Build history of the part. All positions in model axes, mm. Face numbers are marked on the shaded views. A direction names the side the tool comes from. Give positions to 0.01 mm unless a question says otherwise; leave off trailing zeros. Loops run counter-clockwise (first coordinate to the right, second up) from the corner with the lowest first, then second, coordinate; pieces in that order, holes last. Notation, with made-up numbers: (85, 52) -> (141, 52) arc R29 ccw to (141, 81) -> close; hole circle Ø2 at (21, 65.5). An arc over 180 degrees is marked (long way). Answer as a JSON object with one key per item and string values. Group by question number.
Q1. Wall check: probe 1 along X at (y, z) = (-6, 82.5); probe 2 along X at (y, z) = (-10, 86.5). Give the ranges that are in metal, low to high. Write a range as from..to.
Q2. Drop flat-ended pins along their axis: pin 1 (12 mm diameter, centred on y = -4, z = 67.5, fed in from -X); pin 2 (3 mm diameter, centred on y = 5.5, z = 223, fed in from +X); pin 3 (1.2 mm diameter, centred on x = 12, y = -0.5, fed in from +Z). Give the stop position or say it passes through.
Q3. Tool access for the marked faces 1, 2 and 3: list every direction of +Z, -Z, +X, -X, +Y, -Y with a clear straight run to the whole face (end or side of a thin tool).
Q4. Band-saw the part on A-A, the plane z = 61. Write the cut outline in (x, y), plus the area to 3 significant figures.
from build123d import *

# Parameters (mm, degrees)
SKETCH5_OUTSIDE_W  = 88.64
SKETCH5_OUTSIDE_H  = 88.64
CUT_EXTRUDE1_DEPTH = 18
SKETCH6_OUTSIDE_W  = 123.2
SKETCH6_OUTSIDE_H  = 119.18
SKETCH6_OUTSIDE_R  = 12.990381057
CUT_EXTRUDE2_DEPTH = 10
CUT_EXTRUDE2_DRAFT = -60
SKETCH7_OUTSIDE_W  = 123.2
SKETCH7_OUTSIDE_H  = 119.18
SKETCH7_OUTSIDE_R  = 12.990381057
CUT_EXTRUDE3_DEPTH = 10
CUT_EXTRUDE3_DRAFT = -60
SKETCH9_W          = 22
SKETCH9_H          = 25.980762114
CUT_EXTRUDE4_DEPTH = 7
CHAMFER1_SIZE      = 1


with BuildPart() as part:
    # Sketch3 → Revolve1 (revolve)
    with BuildSketch(Plane(origin=(0, 0, 0), x_dir=(0, 0, -1), z_dir=(1, 0, 0)), mode=Mode.PRIVATE) as revolve1_sk:
        Polygon((-38, 12.5), (-38, 0), (-318, 0), (-318, 10), (-299, 10), (-299, 15), (-281, 15), (-281, 10), (-278, 10), (-278, 12.5), align=None)
    revolve(revolve1_sk.sketch.rotate(Axis((0, 0, 318), (0, 0, -1)), 180), axis=Axis((0, 0, 318), (0, 0, -1)))

    # Sketch5 outside → Cut-Extrude1 (cut)
    with BuildSketch(Plane.XY.offset(299)):
        Rectangle(SKETCH5_OUTSIDE_W, SKETCH5_OUTSIDE_H)
        Polygon((7.5, 12.990381057), (-7.5, 12.990381057), (-15, 0), (-7.5, -12.990381057), (7.5, -12.990381057), (15, 0), align=None, mode=Mode.SUBTRACT)
    extrude(amount=-CUT_EXTRUDE1_DEPTH, mode=Mode.SUBTRACT)


with BuildPart() as cut_extrude2_tool:
    # Sketch6 outside → Cut-Extrude2 (with draft: the straight prism first)
    with BuildSketch(Plane.XY.offset(299)):
        Rectangle(SKETCH6_OUTSIDE_W, SKETCH6_OUTSIDE_H)
        Circle(SKETCH6_OUTSIDE_R, mode=Mode.SUBTRACT)
    extrude(amount=-CUT_EXTRUDE2_DEPTH)
    # Cut-Extrude2: the draft: its side faces are tilted about the plane it starts from
    cut_extrude2_sides = [cut_extrude2_tool.faces().sort_by_distance(p)[0] for p in [
        (0, -59.59, 294),
        (61.6, 0, 294),
        (0, 59.59, 294),
        (-61.6, 0, 294),
        (-12.990381057, 0, 294),
    ]]
    draft(cut_extrude2_sides, Plane.XY.offset(299), CUT_EXTRUDE2_DRAFT)


with BuildPart() as part_1:
    add(part.part)

    # Cut-Extrude2: cut by cut_extrude2_tool
    add(cut_extrude2_tool.part, mode=Mode.SUBTRACT)


with BuildPart() as cut_extrude3_tool:
    # Sketch7 outside → Cut-Extrude3 (with draft: the straight prism first)
    with BuildSketch(Plane(origin=(0, 0, 281), x_dir=(-1, 0, 0), z_dir=(0, 0, -1))):
        Rectangle(SKETCH7_OUTSIDE_W, SKETCH7_OUTSIDE_H)
        Circle(SKETCH7_OUTSIDE_R, mode=Mode.SUBTRACT)
    extrude(amount=-CUT_EXTRUDE3_DEPTH)
    # Cut-Extrude3: the draft: its side faces are tilted about the plane it starts from
    cut_extrude3_sides = [cut_extrude3_tool.faces().sort_by_distance(p)[0] for p in [
        (0, -59.59, 286),
        (-61.6, 0, 286),
        (0, 59.59, 286),
        (61.6, 0, 286),
        (12.990381057, 0, 286),
    ]]
    draft(cut_extrude3_sides, Plane(origin=(0, 0, 281), x_dir=(-1, 0, 0), z_dir=(0, 0, -1)), CUT_EXTRUDE3_DRAFT)


with BuildPart() as part_2:
    add(part_1.part)

    # Cut-Extrude3: cut by cut_extrude3_tool
    add(cut_extrude3_tool.part, mode=Mode.SUBTRACT)

    # Sketch9 → Cut-Extrude4 (cut)
    with BuildSketch(Plane.XY.offset(278)):
        with Locations((-22, 0)):
            Rectangle(SKETCH9_W, SKETCH9_H)
        with Locations((22, 0)):
            Rectangle(SKETCH9_W, SKETCH9_H)
    extrude(amount=-CUT_EXTRUDE4_DEPTH, mode=Mode.SUBTRACT)

    # Chamfer1
    chamfer1_edges = [part_2.edges().sort_by_distance(p)[0] for p in [
        (0, 10, 318),
    ]]
    chamfer(chamfer1_edges, length=CHAMFER1_SIZE)


solid = part_2.part
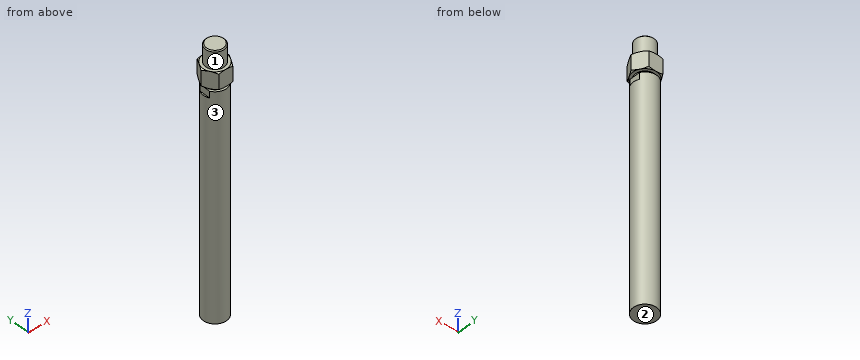
Worked answers:
{
 "1": {"probe 1": "-10.97..10.97", "probe 2": "-7.5..7.5"},
 "2": {"pin 1": "x = -12.5", "pin 2": "x = 11.84", "pin 3": "z = 299"},
 "3": {"face 1": "+Z", "face 2": "-Z, +X, -X, +Y, -Y", "face 3": "-Z"},
 "4": {"outline": "circle Ø25 at (0, 0)", "area": "491 mm2"}
}
